Input: dimensioned drawing with shaded views. Units: mm. Origin: part minimum x, y, z. A direction names the side the tool comes from. Give positions to 0.01 mm unless a question says otherwise; leave off trailing zeros. Order: outer loops, then holes, each group sorted by start corner. A loop starts at its lowest first (then second) coordinate and runs counter-clockwise, first axis right, second up.
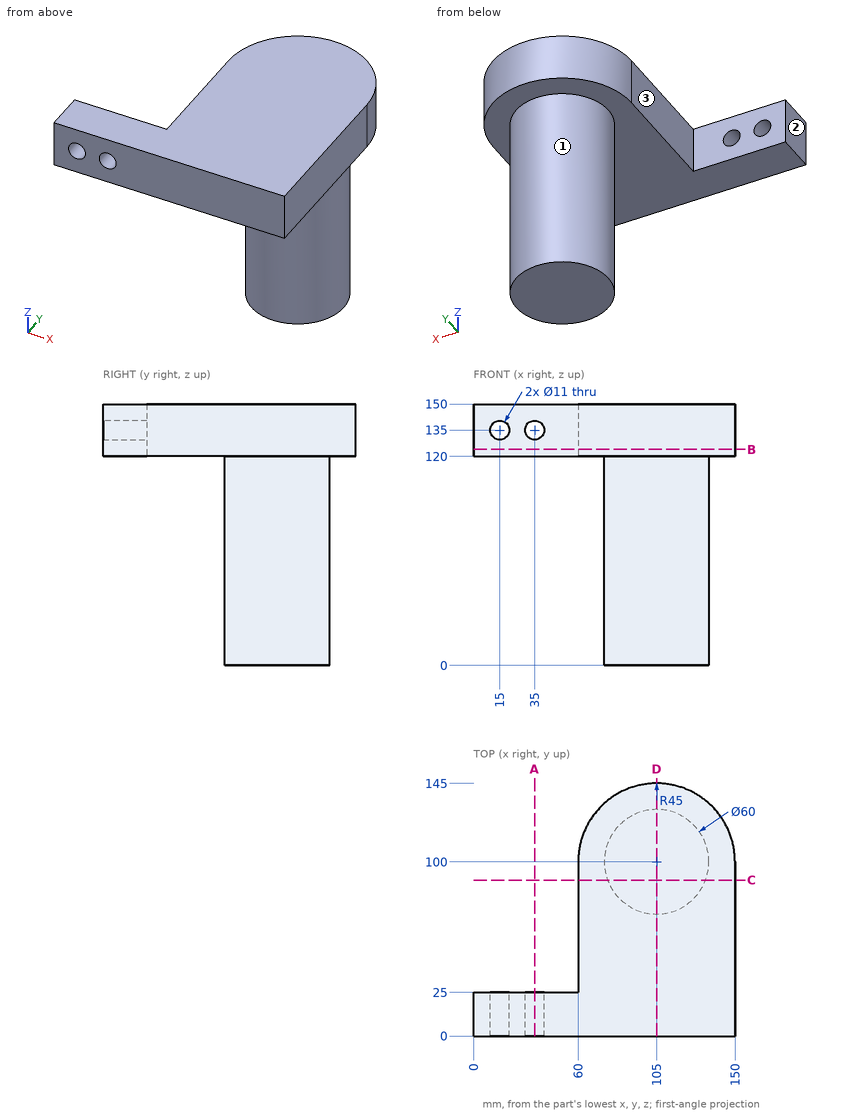
1) Cut plane B-B (z = 124). Return the cut outline in (x, y).
2) First-contact query: P1, Ø9, axis at x = 24, z = 135.5, coming from the +Y side; P2, Ø15, axis at y = 66.5, z = 135.5, coming from the -X side; P3, Ø2, axis at x = 131.5, z = 61, coming from the +Y side. Flat tips, straight axial feed; report the tip coordinate or a pass-through.
3) Reachability of the marked faces 1, 2 and 3 from +Z, -Z, +X, -X, +Y, -Y: full face, straight path, thin tool, end or side. Return the list, or none.
4) Cut plane D-D (x = 105). Return the cut outline in (y, z), then the cut area to 4 significant figures.
5) Cut plane C-C (y = 89.5). Return the cut outline in (x, z).
6) Line query: probe 1 along X at (y, z) = (19, 135); probe 2 along Z at (x, y) = (139.5, 79); probe 3 along Y at (x, z) = (111, 65.5). Output: solid intervals per line, ascending.
7) Cut plane A-A (x = 35). Return the cut outline in (y, z).
Geometry says:
1. outline: (0, 0) - (150, 0) - (150, 100) arc R45 ccw to (60, 100) - (60, 25) - (0, 25) - close
2. P1: stops at y = 25
2. P2: stops at x = 60
2. P3: stops at y = 115.8
3. face 1: -Z
3. face 2: +Z, -Z, -X, +Y, -Y
3. face 3: +Z, -Z, -X, +Y
4. outline: (0, 120) - (70, 120) - (70, 0) - (130, 0) - (130, 120) - (145, 120) - (145, 150) - (0, 150) - close
4. area: 11,550 mm2
5. outline: (60, 120) - (76.9, 120) - (76.9, 0) - (133.1, 0) - (133.1, 120) - (150, 120) - (150, 150) - (60, 150) - close
6. probe 1: x = 0 to 9.5, 20.5 to 29.5, 40.5 to 150
6. probe 2: z = 120 to 150
6. probe 3: y = 70.61 to 129.39
7. outline: (0, 120) - (25, 120) - (25, 129.5) - (0, 129.5) - close; (0, 140.5) - (25, 140.5) - (25, 150) - (0, 150) - close
